The drawing under review shows one solid part. Ordinate dimensions are in mm from its lowest x, y, z. A direction names the side the tool comes from. Give positions to 0.01 mm unless a question says otherwise; leave off trailing zeros. Loops run counter-clockwise (first coordinate to the right, second up) from the corner with the lowest first, then second, coordinate; pieces in that order, holes last. Notation, with made-up numbers: (-31.75, 7) -> (13.25, 7) arc R26 ccw to (13.25, 31) -> close; hole circle Ø11 at (70, 20). An arc over 180 degrees is marked (long way). Answer in a Markdown table with one row per item. Add a question column.
(1) Consider section D-D on x = 35. Write out the cut boundary in (y, z).
(2) For line 1 (Y direction, x = 55, z = 93.5); line 2 (X direction, y = 73.3, z = 25); line 3 (Z direction, x = 35.5, y = 22), list the stretches that pass through material, from the lowest coordinate up.
(3) Draft analysis for pull direction X (two halves, no side actions). For the marked faces 1, 2, 3 and 4, state which applies: +X half, -X half, draft (parallel to the pull), parting line (faces both ways), or undercut.
(4) Consider section A-A on x = 55. Write out the cut boundary in (y, z).
(5) For pin 1 (14 mm diameter, centred on x = 15, y = 45, fed in from -Z); pin 2 (5.5 mm diameter, centred on y = 71.5, z = 57.5, fed in from +X); pin 3 (12 mm diameter, centred on x = 48.5, z = 58.5, fed in from -Y), all flat-tipped, find the tip position at first contact; note any pin that passes through.
(6) For the marked faces 5 and 6, list the 3-axis set-ups (+Z, -Z, +X, -X, +Y, -Y) from which the entire face can be reached by the end or side of a thin tool; tool diameter is ignored.
(7) Consider section C-C on z = 94.5. Write out the cut boundary in (x, y), then the cut area to 3 significant figures.
(8) Consider section B-B on y = 45. Write out the cut boundary in (x, z), then the cut area to 3 significant figures.
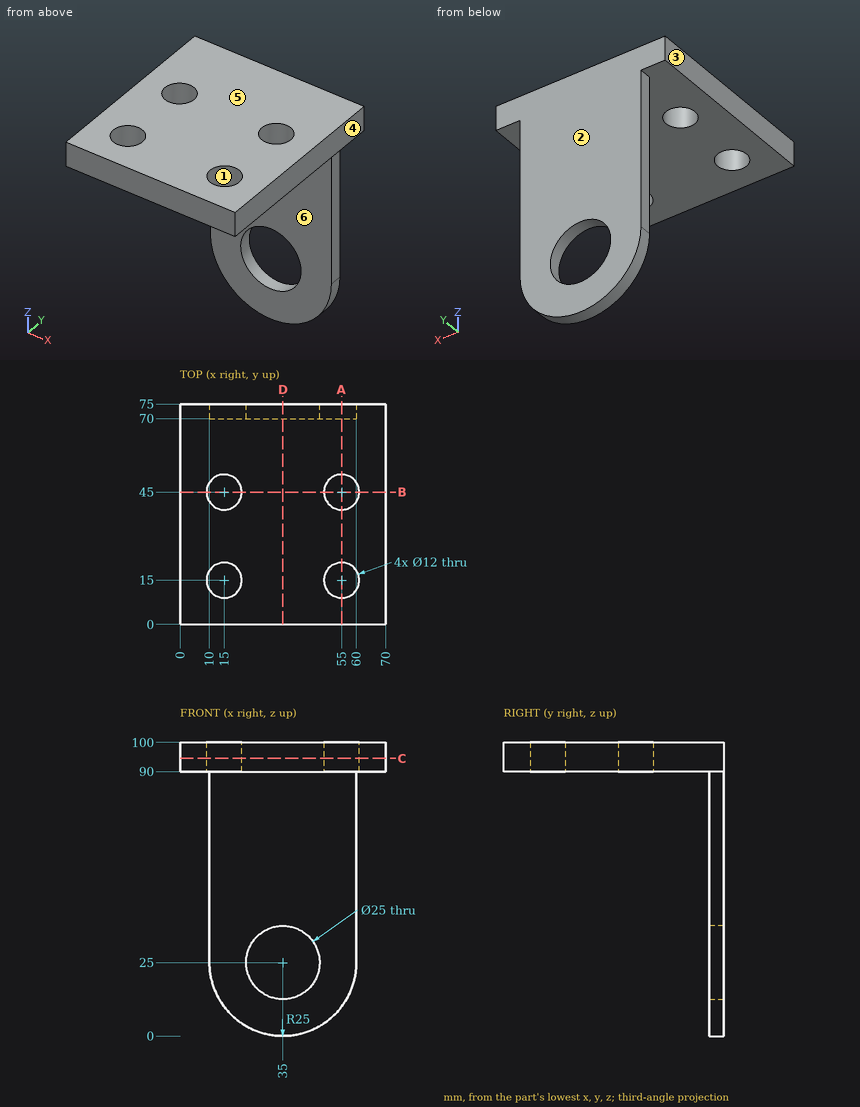
Values follow:
| question | item | result |
|---|---|---|
| 1 | outline | (0, 90) -> (70, 90) -> (70, 37.5) -> (75, 37.5) -> (75, 100) -> (0, 100) -> close; (70, 0) -> (75, 0) -> (75, 12.5) -> (70, 12.5) -> close |
| 2 | line 1 | 0 to 9, 21 to 39, 51 to 75 |
| 2 | line 2 | 10 to 22.5, 47.5 to 60 |
| 2 | line 3 | 90 to 100 |
| 3 | face 1 | undercut |
| 3 | face 2 | draft |
| 3 | face 3 | -X half |
| 3 | face 4 | +X half |
| 4 | outline | (0, 90) -> (9, 90) -> (9, 100) -> (0, 100) -> close; (21, 90) -> (39, 90) -> (39, 100) -> (21, 100) -> close; (51, 90) -> (70, 90) -> (70, 10) -> (75, 10) -> (75, 100) -> (51, 100) -> close |
| 5 | pin 1 | z = 90 |
| 5 | pin 2 | x = 60 |
| 5 | pin 3 | y = 70 |
| 6 | face 5 | +Z, +X, -X, +Y, -Y |
| 6 | face 6 | -Z, +X, -X, -Y |
| 7 | outline | (0, 0) -> (70, 0) -> (70, 75) -> (0, 75) -> close; hole circle Ø12 at (15, 15); hole circle Ø12 at (15, 45); hole circle Ø12 at (55, 15); hole circle Ø12 at (55, 45) |
| 7 | area | 4,800 mm2 |
| 8 | outline | (0, 90) -> (9, 90) -> (9, 100) -> (0, 100) -> close; (21, 90) -> (49, 90) -> (49, 100) -> (21, 100) -> close; (61, 90) -> (70, 90) -> (70, 100) -> (61, 100) -> close |
| 8 | area | 460 mm2 |
